For this review, take the finished solid that the model builds, in its own axes (mm). Face numbers are marked on the shaded views. A direction names the side the tool comes from. Give positions to 0.01 mm unless a question says otherwise; leave off trailing zeros. Order: outer loops, then holes, each group sorted by start corner. A loop starts at its lowest first (then second) coordinate and runs counter-clockwise, first axis right, second up.
from build123d import *

# Parameters (mm, degrees)
SKETCH_2_R          = 15
CUT_EXTRUDE_1_DEPTH = 50
CUT_EXTRUDE_START   = -7.5
SKETCH_3_W          = 8
SKETCH_3_H          = 7
CUT_EXTRUDE_2_DEPTH = 512.59
CUT_EXTRUDE_3_DEPTH = 7


with BuildPart() as part:
    # 草图1 → 旋转1 (revolve)
    with BuildSketch(Plane.XY, mode=Mode.PRIVATE) as revolve_1_sk:
        Polygon((0, -243.614201173), (15, -243.614201173), (15, -208.614201173), (10, -208.614201173), (10, -203.614201173), (20, -203.614201173), (20, -174.914201173), (18, -174.914201173), (18, -171.914201173), (20, -171.914201173), (20, -118.614201173), (40, -118.614201173), (40, -93.614201173), (30, -93.614201173), (30, 461.975798827), (0, 461.975798827), align=None)
    revolve(revolve_1_sk.sketch.rotate(Axis((0, 247.860200322, 0), (0, -1, 0)), 90), axis=Axis((0, 247.860200322, 0), (0, -1, 0)))

    # 草图2 → 切除-拉伸1 (cut)
    with BuildSketch(Plane(origin=(0, 461.975798827, 0), x_dir=(1, 0, 0), z_dir=(0, 1, 0))):
        with Locations(Location((0, 0, 0), (0, 0, 270))):
            Circle(SKETCH_2_R)
    extrude(amount=-CUT_EXTRUDE_1_DEPTH, mode=Mode.SUBTRACT)

    # 草图3 → 切除-拉伸2 (cut)
    with BuildSketch(Plane(origin=(0, 461.975798827, 0), x_dir=(1, 0, 0), z_dir=(0, 1, 0)).offset(CUT_EXTRUDE_START)):
        with Locations((0, -29.732137495)):
            Rectangle(SKETCH_3_W, SKETCH_3_H)
    extrude(amount=-CUT_EXTRUDE_2_DEPTH, mode=Mode.SUBTRACT)

    # 草图4 → 切除-拉伸3 (cut)
    with BuildSketch(Plane.XY.offset(26.232137495)):
        with BuildLine():
            Line((4, -58.114201173), (-4, -58.114201173))
            ThreePointArc((-4, -58.114201173), (0, -62.114201173), (4, -58.114201173))
        make_face()
        with BuildLine():
            Line((-4, 454.475798827), (4, 454.475798827))
            ThreePointArc((4, 454.475798827), (0, 458.475798827), (-4, 454.475798827))
        make_face()
    extrude(amount=CUT_EXTRUDE_3_DEPTH, mode=Mode.SUBTRACT)


solid = part.part
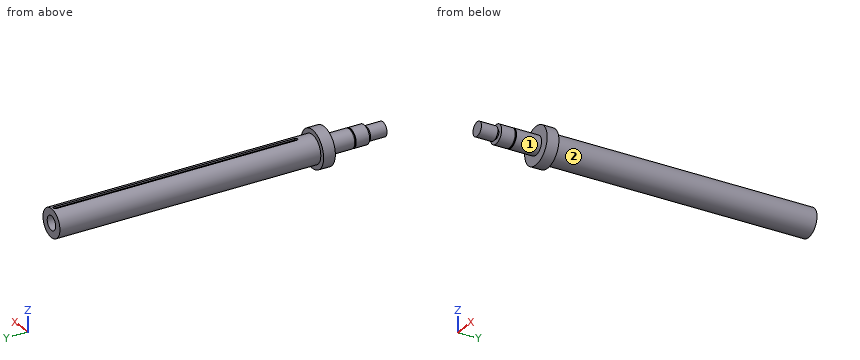
1) Tool access review of the marked faces 1 and 2: name each direction out of +Z, -Z, +X, -X, +Y, -Y from which nothing blocks a thin tool from reaching the whole face with its end or side.
Answer sheet:
face 1: -Y
face 2: +Y
2) To check wall thickness, follow line 1 (X direction, y = 434, z = 0); line 2 (Y direction, x = -11, z = 13); line 3 (Y direction, x = 32.5, z = -13.5). State the ranges of each line that lie inside material, in increasing order.
Answer sheet:
line 1: x = -30 to -15, 15 to 30
line 2: y = -203.61 to 461.98
line 3: y = -118.61 to -93.61
3) Clearance check with flat-ended pins moving along their axes: pin 1 (8 mm diameter, centred on x = -24, y = -27, fed in from -Z); pin 2 (3 mm diameter, centred on y = 197, z = -10, fed in from +X); pin 3 (2 mm diameter, centred on y = 133, z = 21.5, fed in from +X); pin 4 (1.5 mm diameter, centred on y = 226.5, z = 31, fed in from +X). State where each tip first meets the part, or that it passes through.
Answer sheet:
pin 1: stops at z = -22.36
pin 2: stops at x = 28.77
pin 3: stops at x = 21.9
pin 4: passes through
4) We need section B-B on y = 376. Give the boundary of the cut face in (x, z), then the cut area to 3 significant figures.
Answer sheet:
outline: (-4, 26.23) - (-4, 29.73) arc R30 ccw (long way) to (4, 29.73) - (4, 26.23) - close
area: 2,800 mm2
